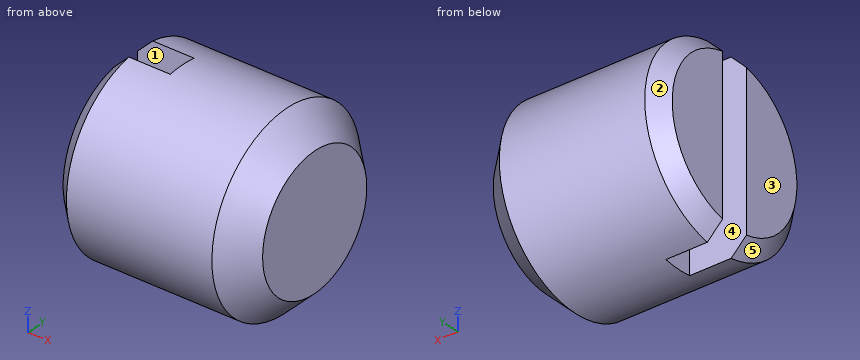
from build123d import *

# Parameters (mm, degrees)
NOTCH_DEPTH      = 13.247448714
NOTCH_DEPTH_BACK = 13.247448714
SKETCH2_W        = 3
SKETCH2_H        = 1.6


with BuildPart() as part:
    # Sketch1 → Base (revolve)
    with BuildSketch(Plane.XY, mode=Mode.PRIVATE) as base_sk:
        Polygon((0, 0), (10, 0), (10, 3.5), (8.5, 5), (0.812, 5), (0, 4.188), align=None)
    revolve(base_sk.sketch.rotate(Axis((-10.745014543, 0, 0), (1, 0, 0)), 90), axis=Axis((-10.745014543, 0, 0), (1, 0, 0)))

    # Sketch2 → Notch (cut, two sides: drawn at the far end of the back side and taken through both)
    with BuildSketch(Plane.XY.offset(-NOTCH_DEPTH_BACK)):
        with Locations((1.5, 0)):
            Rectangle(SKETCH2_W, SKETCH2_H)
    extrude(amount=NOTCH_DEPTH + NOTCH_DEPTH_BACK, mode=Mode.SUBTRACT)


solid = part.part
Work out the finished part from the listing and answer in its coordinate system (mm). Face numbers are marked on the shaded views. A direction names the side the tool comes from. Round coordinates to 2 decimals unless told otherwise and drop trailing zeros. Write each loop counter-clockwise with the first axis right and the second up, starting at its lowest first coordinate (ties: lowest second). Pieces come first, ordered by that corner, then holes.
1) A tool of negligible diameter and unlimited length cuts with its end or side. For the marked faces 1 and 2, from which of +Z, -Z, +X, -X, +Y, -Y can it reach the whole face along a straight path? Write none if from no direction.
2) A cutting plane is placed at C-C (y = 0). Give the vertices of the cut face in (x, z), plus the area to 4 significant figures.
3) A cutting plane is placed at A-A (z = 0). Give the vertices of the cut face in (x, y).
4) Straight lines are drawn through the part: line 1 (Y direction, x = 1.5, z = 1.5); line 2 (X direction, y = -2.75, z = -4); line 3 (Z direction, x = 7.25, y = -2.75). For each, find the intervals that lie inside material, in ascending order.
5) A cutting plane is placed at B-B (x = 7.75). Give the vertices of the cut face in (y, z), plus the area to 3 significant figures.
6) Given pin 1 Ø2.5 at (x, z) = (1, 1.5) entering from -Y; pin 2 Ø1.5 at (y, z) = (-2.5, 3.5) entering from +X; pin 3 Ø0.5 at (y, z) = (-0.5, 0.5) entering from -X, each flat-ended and moving along its own axis, determine where each tip first touches the part or whether it passes through.
7) The mould has two halves that part along Y. Classify the marked faces 3, 4 and 5: pulls with the +Y half, pulls with the -Y half, needs draft (parallel to the pull), parting line crosses it, or undercut.
Completed:
1. face 1: +Z, -Z, -X
1. face 2: -X, +Y
2. outline: (3, -5) - (8.5, -5) - (10, -3.5) - (10, 3.5) - (8.5, 5) - (3, 5) - close
2. area: 67.75 mm2
3. outline: (0, -4.19) - (0.81, -5) - (8.5, -5) - (10, -3.5) - (10, 3.5) - (8.5, 5) - (0.81, 5) - (0, 4.19) - (0, 0.8) - (3, 0.8) - (3, -0.8) - (0, -0.8) - close
4. line 1: y = -4.77 to -0.8, 0.8 to 4.77
4. line 2: x = 0.67 to 8.65
4. line 3: z = -4.18 to 4.18
5. outline: circle Ø10 at (0, 0)
5. area: 78.5 mm2
6. pin 1: stops at y = -4.99
6. pin 2: stops at x = 9.95
6. pin 3: stops at x = 3
7. face 3: needs draft
7. face 4: undercut
7. face 5: pulls with the -Y half
